from build123d import *

# Parameters (mm, degrees)
BOSS_EXTRUDE1_DEPTH = 1110


with BuildPart() as part:
    # Sketch1 → Boss-Extrude1 (new body)
    with BuildSketch(Plane.XY):
        with BuildLine():
            Line((0, 0), (65, 0))
            ThreePointArc((65, 0), (72.071067812, -2.928932188), (75, -10))
            Line((75, -10), (75, -40))
            Line((75, -40), (69, -40))
            Line((69, -40), (69, -10))
            ThreePointArc((69, -10), (67.828427125, -7.171572875), (65, -6))
            Line((65, -6), (0, -6))
            Line((0, -6), (0, 0))
        make_face()
    extrude(amount=BOSS_EXTRUDE1_DEPTH)


solid = part.part
Read the model definition and answer for the solid it produces. Units are mm, in the model's axes. A direction names the side the tool comes from. Give positions to 0.01 mm unless a question says otherwise; leave off trailing zeros. Loops run counter-clockwise (first coordinate to the right, second up) from the corner with the lowest first, then second, coordinate; pieces in that order, holes last. Notation, with made-up numbers: (78, 25) - (88, 25) arc R21 ccw to (88, 59) - close; hole circle Ø2 at (-5.75, 72.5). An arc over 180 degrees is marked (long way). Answer as CSV lines item,"result". Start each with the question number.
1) Straight lines are drawn through the part: L1, parallel to Y at x = 49.5, z = 542; L2, parallel to X at y = -34, z = 700; L3, parallel to Y at x = 66, z = 1030.5. For each, find the intervals that lie inside material, in ascending order. Write a range as from..to.
2) Find section A-A (z = 835). Write down the section's boundary in (x, y).
3) This flat-tipped pin is pushed along its axis until it touches: pin 1 Ø6 at (y, z) = (-34, 702.5) entering from -X. Where does it stop, or does it pass through?
4) Find section B-B (y = -28). Write down the section's boundary in (x, z), then the cut area to 3 significant figures.
5) Find section C-C (x = 22.5). Write down the section's boundary in (y, z), then the cut area to 3 significant figures.
6) Which of the six approach directions +Z, -Z, +X, -X, +Y, -Y give full straight-line access (tool end or side, diameter ignored) to faces 1 (the face through (33, -6, 547)), 2 (the face through (75, -25, 547))?
Findings below:
1,L1,"-6..0"
1,L2,"69..75"
1,L3,"-6.13..-0.05"
2,outline,"(0, -6) - (65, -6) arc R4 cw to (69, -10) - (69, -40) - (75, -40) - (75, -10) arc R10 ccw to (65, 0) - (0, 0) - close"
3,pin 1,"x = 69"
4,outline,"(69, 0) - (75, 0) - (75, 1110) - (69, 1110) - close"
4,area,"6,660 mm^2"
5,outline,"(-6, 0) - (0, 0) - (0, 1110) - (-6, 1110) - close"
5,area,"6,660 mm^2"
6,face 1,"+Z, -Z, -X, -Y"
6,face 2,"+Z, -Z, +X, +Y, -Y"
